```python
from build123d import *

# Parameters (mm, degrees)
EXTRUDE_THIN1_DEPTH = 2
BOSS_EXTRUDE1_DEPTH = 28
CUT_EXTRUDE1_DEPTH  = 28


with BuildPart() as part:
    # Sketch1 → Extrude-Thin1 (new body)
    with BuildSketch(Plane.XY):
        with BuildLine():
            Line((0, 0), (0, 40))
            ThreePointArc((0, 40), (-2.928932188, 47.071067812), (-10, 50))
            Line((-10, 50), (-30, 50))
            Line((-30, 50), (-30, 65))
            Line((-30, 65), (-10, 65))
            ThreePointArc((-10, 65), (7.67766953, 57.67766953), (15, 40))
            Line((15, 40), (15, 0))
            Line((15, 0), (0, 0))
        make_face()
    extrude(amount=EXTRUDE_THIN1_DEPTH)

    # Sketch2 → Boss-Extrude1 (add)
    with BuildSketch(Plane.XY.offset(2)):
        with BuildLine():
            Line((13, 0), (13, 40))
            ThreePointArc((13, 40), (6.263455967, 56.263455967), (-10, 63))
            Line((-10, 63), (-30, 63))
            Line((-30, 63), (-30, 65))
            Line((-30, 65), (-10, 65))
            ThreePointArc((-10, 65), (7.67766953, 57.67766953), (15, 40))
            Line((15, 40), (15, 0))
            Line((15, 0), (13, 0))
        make_face()
    extrude(amount=BOSS_EXTRUDE1_DEPTH)

    # Sketch3 → Cut-Extrude1 (cut)
    with BuildSketch(Plane.XY.offset(2)):
        with BuildLine():
            Line((-19.283890524, 59.176308794), (-19.283890524, 52.835918308))
            ThreePointArc((-19.283890524, 52.835918308), (-21.035277496, 51.084531336), (-22.786664469, 52.835918308))
            Line((-22.786664469, 52.835918308), (-22.786664469, 59.176308794))
            ThreePointArc((-22.786664469, 59.176308794), (-21.035277496, 60.927695767), (-19.283890524, 59.176308794))
        make_face()
        with BuildLine():
            Line((3.842402099, 13.695706596), (8.588468352, 13.695706596))
            ThreePointArc((8.588468352, 13.695706596), (10.164668971, 12.119505978), (8.588468352, 10.543305359))
            Line((8.588468352, 10.543305359), (3.842402099, 10.543305359))
            ThreePointArc((3.842402099, 10.543305359), (2.26620148, 12.119505978), (3.842402099, 13.695706596))
        make_face()
        with BuildLine():
            Line((3.842402099, 37.707268764), (8.588468352, 37.707268764))
            ThreePointArc((8.588468352, 37.707268764), (10.388432438, 35.907304678), (8.588468352, 34.107340593))
            Line((8.588468352, 34.107340593), (3.842402099, 34.107340593))
            ThreePointArc((3.842402099, 34.107340593), (2.042438013, 35.907304678), (3.842402099, 37.707268764))
        make_face()
    extrude(amount=-CUT_EXTRUDE1_DEPTH, mode=Mode.SUBTRACT)


solid = part.part
```
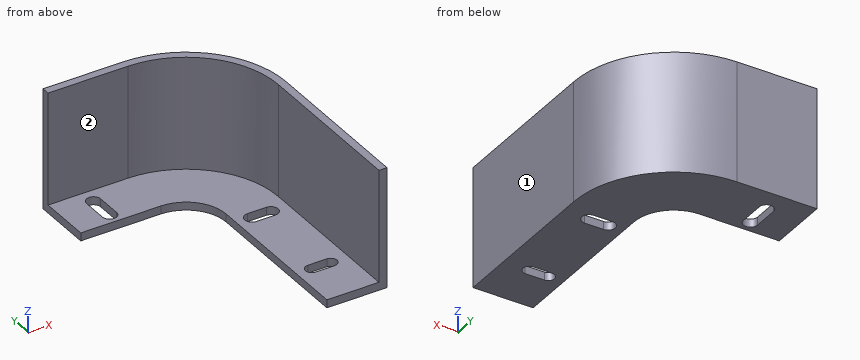
The model under review builds one solid part; all positions refer to its coordinate system, in mm. Face numbers are marked on the shaded views. A direction names the side the tool comes from. Give positions to 0.01 mm unless a question says otherwise; leave off trailing zeros. Loops run counter-clockwise (first coordinate to the right, second up) from the corner with the lowest first, then second, coordinate; pieces in that order, holes last. Notation, with made-up numbers: (58, 48) -> (89, 48) arc R28 ccw to (89, 83) -> close; hole circle Ø3 at (-35, 29). An arc over 180 degrees is marked (long way). Use CSV: the item, a comma, the result in double quotes.
1. Consider section D-D, the plane x = -20. Write out the cut boundary in (y, z), then the cut area to 3 significant figures.
Result:
outline,"(50, 0) -> (51.42, 0) -> (51.42, 2) -> (50, 2) -> close; (60.59, 0) -> (65, 0) -> (65, 30) -> (63, 30) -> (63, 2) -> (60.59, 2) -> close"
area,"67.7 mm²"
2. Consider section A-A, the plane x = 6. Write out the cut boundary in (y, z), then the cut area to 3 significant figures.
Result:
outline,"(0, 0) -> (10.54, 0) -> (10.54, 2) -> (0, 2) -> close; (13.7, 0) -> (34.11, 0) -> (34.11, 2) -> (13.7, 2) -> close; (37.71, 0) -> (59.21, 0) -> (59.21, 30) -> (56.52, 30) -> (56.52, 2) -> (37.71, 2) -> close"
area,"180 mm²"
3. Machinability: for the marked faces 1 and 2, which of the approach directions +Z, -Z, +X, -X, +Y, -Y give a long, thin tool a straight path to every point of the face, cutting with its end or side? Answer none if there is none.
Result:
face 1,"+Z, -Z, +X, +Y, -Y"
face 2,"+Z, -X, -Y"
4. Consider section C-C, the plane y = 35.5. Write out the cut boundary in (x, z), then the cut area to 3 significant figures.
Result:
outline,"(0, 0) -> (2.09, 0) -> (2.09, 2) -> (0, 2) -> close; (10.34, 0) -> (15, 0) -> (15, 30) -> (13, 30) -> (13, 2) -> (10.34, 2) -> close"
area,"69.5 mm²"
5. To check wall thickness, follow probe 1 along Y at (x, z) = (3, 1.25); probe 2 along Y at (x, z) = (-16.5, 7.75); probe 3 along X at (y, z) = (16, 16.5). State the ranges of each line that lie inside material, in increasing order. Write a range as from..to.
Result:
probe 1,"y = 0..10.79, 13.45..34.32, 37.5..61.35"
probe 2,"y = 63..65"
probe 3,"x = 13..15"
6. Consider section B-B, the plane z = 5.25. Write out the cut boundary in (x, y).
Result:
outline,"(-30, 63) -> (-10, 63) arc R23 cw to (13, 40) -> (13, 0) -> (15, 0) -> (15, 40) arc R25 ccw to (-10, 65) -> (-30, 65) -> close"
7. For P1, Ø0.6, axis at x = 6.5, z = 1, coming from the -Y side; P2, Ø2, axis at x = 6, z = 1, coming from the +Y side; P3, Ø4, axis at y = 44.5, z = 22, coming from the -X side; P4, Ø13, axis at x = -1, y = 35.5, coming from the +Z side, all flat-tipped, find the tip position at first contact; note any pin that passes through.
Result:
P1,"stops at y = 0"
P2,"stops at y = 60"
P3,"stops at x = 12.06"
P4,"stops at z = 2"
